Geometry check sheet. Reference: the model listing, model coordinates, mm. Coordinates: 2 decimals unless noted, no trailing zeros. Order: outer loops, then holes, each group sorted by start corner. A loop starts at its lowest first (then second) coordinate and runs counter-clockwise, first axis right, second up. Notation, with made-up numbers: (15.25, 77.5) -> (38.25, 77.5) arc R13 cw to (38.25, 93.5) -> close; hole circle Ø10 at (30.25, 40.25). An arc over 180 degrees is marked (long way). Answer in a Markdown table with one row per item. Add a question column.
```python
from build123d import *

# Parameters (mm, degrees)
WEB_DISC_PROFILE_90_R                  = 44
WEB_DISC_90X5_DEPTH                    = 5
BORE_AND_SPOKE_WINDOWS_PROFILE_R       = 14.25
CENTRE_BORE_AND_4X_SPOKE_WINDOWS_DEPTH = 44


with BuildPart() as part:
    # Web Disc Profile Ø90 → Web Disc Ø90x5 (new body)
    with BuildSketch(Plane(origin=(0, 0, 0), x_dir=(1, 0, 0), z_dir=(0, 1, 0))):
        with Locations(Location((0, 0, 0), (0, 0, 270))):
            Circle(WEB_DISC_PROFILE_90_R)
    extrude(amount=WEB_DISC_90X5_DEPTH)

    # Bore and Spoke Windows Profile → Centre Bore and 4x Spoke Windows (cut)
    with BuildSketch(Plane(origin=(0, 5, 0), x_dir=(1, 0, 0), z_dir=(0, 1, 0))):
        with BuildLine():
            Line((-21.966508598, 6.35), (-33.801294354, 6.35))
            ThreePointArc((-33.801294354, 6.35), (-37.437163198, 8.198498964), (-38.085965469, 12.225352113))
            ThreePointArc((-38.085965469, 12.225352113), (-28.284271247, 28.284271247), (-12.225352113, 38.085965469))
            ThreePointArc((-12.225352113, 38.085965469), (-8.198498964, 37.437163198), (-6.35, 33.801294354))
            Line((-6.35, 33.801294354), (-6.35, 21.966508598))
            ThreePointArc((-6.35, 21.966508598), (-7.027837187, 19.591414615), (-8.857142857, 17.931843754))
            ThreePointArc((-8.857142857, 17.931843754), (-14.142135624, 14.142135624), (-17.931843754, 8.857142857))
            ThreePointArc((-17.931843754, 8.857142857), (-19.591414615, 7.027837187), (-21.966508598, 6.35))
        make_face()
        with BuildLine():
            Line((21.966508598, 6.35), (33.801294354, 6.35))
            ThreePointArc((33.801294354, 6.35), (37.437163198, 8.198498964), (38.085965469, 12.225352113))
            ThreePointArc((38.085965469, 12.225352113), (28.284271247, 28.284271247), (12.225352113, 38.085965469))
            ThreePointArc((12.225352113, 38.085965469), (8.198498964, 37.437163198), (6.35, 33.801294354))
            Line((6.35, 33.801294354), (6.35, 21.966508598))
            ThreePointArc((6.35, 21.966508598), (7.027837187, 19.591414615), (8.857142857, 17.931843754))
            ThreePointArc((8.857142857, 17.931843754), (14.142135624, 14.142135624), (17.931843754, 8.857142857))
            ThreePointArc((17.931843754, 8.857142857), (19.591414615, 7.027837187), (21.966508598, 6.35))
        make_face()
        with BuildLine():
            Line((21.966508598, -6.35), (33.801294354, -6.35))
            ThreePointArc((33.801294354, -6.35), (37.437163198, -8.198498964), (38.085965469, -12.225352113))
            ThreePointArc((38.085965469, -12.225352113), (28.284271247, -28.284271247), (12.225352113, -38.085965469))
            ThreePointArc((12.225352113, -38.085965469), (8.198498964, -37.437163198), (6.35, -33.801294354))
            Line((6.35, -33.801294354), (6.35, -21.966508598))
            ThreePointArc((6.35, -21.966508598), (7.027837187, -19.591414615), (8.857142857, -17.931843754))
            ThreePointArc((8.857142857, -17.931843754), (14.142135624, -14.142135624), (17.931843754, -8.857142857))
            ThreePointArc((17.931843754, -8.857142857), (19.591414615, -7.027837187), (21.966508598, -6.35))
        make_face()
        with BuildLine():
            Line((-6.35, -21.966508598), (-6.35, -33.801294354))
            ThreePointArc((-6.35, -33.801294354), (-8.198498964, -37.437163198), (-12.225352113, -38.085965469))
            ThreePointArc((-12.225352113, -38.085965469), (-28.284271247, -28.284271247), (-38.085965469, -12.225352113))
            ThreePointArc((-38.085965469, -12.225352113), (-37.437163198, -8.198498964), (-33.801294354, -6.35))
            Line((-33.801294354, -6.35), (-21.966508598, -6.35))
            ThreePointArc((-21.966508598, -6.35), (-19.591414615, -7.027837187), (-17.931843754, -8.857142857))
            ThreePointArc((-17.931843754, -8.857142857), (-14.142135624, -14.142135624), (-8.857142857, -17.931843754))
            ThreePointArc((-8.857142857, -17.931843754), (-7.027837187, -19.591414615), (-6.35, -21.966508598))
        make_face()
        with Locations(Location((0, 0, 0), (0, 0, 270))):
            Circle(BORE_AND_SPOKE_WINDOWS_PROFILE_R)
    extrude(amount=-CENTRE_BORE_AND_4X_SPOKE_WINDOWS_DEPTH, mode=Mode.SUBTRACT)


solid = part.part
```
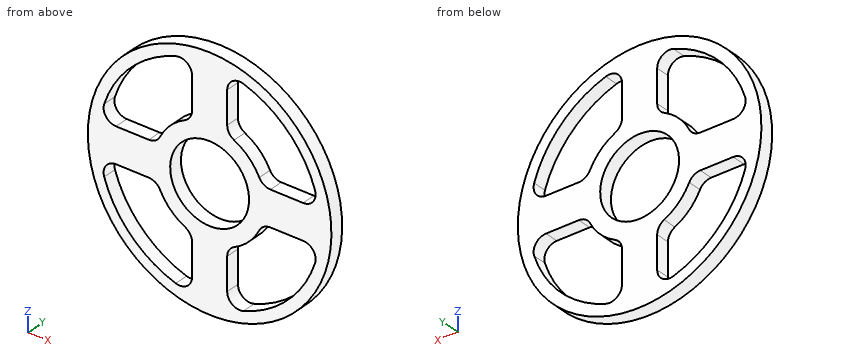
(1) Cross-section at A-A (x = 0). Enter the section's corners in (y, z), plus the area to 4 significant figures.
(2) Go/stop test with flat-tipped pins: P1, Ø2.5, axis at x = -26.5, y = 2.5, coming from the -Z side; P2, Ø1, axis at y = 1.5, z = 23.5, coming from the +X side; P3, Ø1.5, axis at y = 2, z = 30, coming from the -X side; P4, Ø10, axis at x = 4, z = 27.5, coming from the -Y side. Record where each tip stops, or that it passes through.
(3) Cross-section at B-B (y = 3.6). Give the number of separate pieces and of enclosed holes in the cut face, plus the area to 3 significant figures.
(4) Cross-section at D-D (x = -26.5). Enter the section's corners in (y, z), plus the area to 3 significant figures.
(5) Cross-section at C-C (z = 0). Enter the section's corners in (x, y).
(6) Scan lines: line 1 along X through (y, z) = (1.25, 16); line 2 along Z through (x, y) = (-11, 4.75); line 3 along X through (y, z) = (4.5, 35). Record each from-to range of solid material in increasing order.
Checks:
| question | item | result |
|---|---|---|
| 1 | outline | (0, -44) -> (5, -44) -> (5, -14.25) -> (0, -14.25) -> close; (0, 14.25) -> (5, 14.25) -> (5, 44) -> (0, 44) -> close |
| 1 | area | 297.5 mm² |
| 2 | P1 | z = -36.03 |
| 2 | P2 | x = 37.51 |
| 2 | P3 | x = -32.87 |
| 2 | P4 | y = 0 |
| 3 | separate pieces | 1 |
| 3 | enclosed holes | 5 |
| 3 | area | 2,770 mm² |
| 4 | outline | (0, -35.12) -> (5, -35.12) -> (5, -29.96) -> (0, -29.96) -> close; (0, -6.35) -> (5, -6.35) -> (5, 6.35) -> (0, 6.35) -> close; (0, 29.96) -> (5, 29.96) -> (5, 35.12) -> (0, 35.12) -> close |
| 4 | area | 115 mm² |
| 5 | outline | (-44, 0) -> (-14.25, 0) -> (-14.25, 5) -> (-44, 5) -> close; (14.25, 0) -> (44, 0) -> (44, 5) -> (14.25, 5) -> close |
| 6 | line 1 | -40.99 to -36.66, -12 to 12, 36.66 to 40.99 |
| 6 | line 2 | -42.6 to -38.3, -16.7 to -9.06, 9.06 to 16.7, 38.3 to 42.6 |
| 6 | line 3 | -26.66 to -19.36, -6.51 to 6.51, 19.36 to 26.66 |
